Can you work these out from the drawing? Everything is in mm from the part's minimum corner. A direction names the side the tool comes from. Round coordinates to 2 decimals unless told otherwise and drop trailing zeros. Order: outer loops, then holes, each group sorted by start corner. A loop starts at its lowest first (then second) coordinate and runs counter-clockwise, first axis right, second up. Notation, with made-up numbers: (37.5, 69.5) - (56.5, 69.5) arc R29 ccw to (56.5, 104.5) - close; hole circle Ø10 at (-8, -18.5). An arc over 180 degrees is marked (long way). Write item = value, one per line.
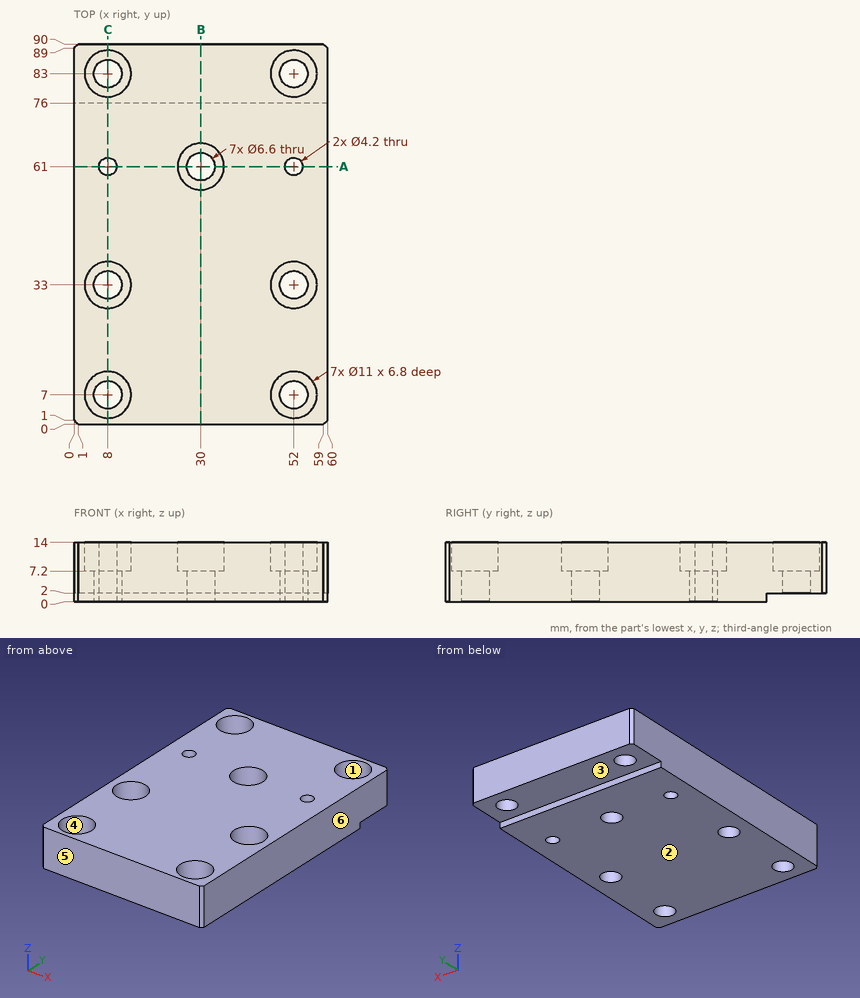
(1) If we section it at B-B (x = 30): Write out the boundary of the cut face in (y, z).
Computed:
outline = (0, 0) - (57.7, 0) - (57.7, 7.2) - (55.5, 7.2) - (55.5, 14) - (0, 14) - close; (64.3, 0) - (76, 0) - (76, 2) - (90, 2) - (90, 14) - (66.5, 14) - (66.5, 7.2) - (64.3, 7.2) - close
(2) Will these pins go through, and if not, where does the flat tip stop? P1, Ø12, axis at x = 32.5, y = 61.5, coming from the +Z side; P2, Ø7.5, axis at x = 52, y = 83, coming from the +Z side; P3, Ø0.6, axis at x = 32, z = 0.5, coming from the +Y side.
Computed:
P1 = 14
P2 = 7.2
P3 = 76
(3) On a 3-axis mill with a long thin cutter (end or side, diameter ignored), from which of +Z, -Z, +X, -X, +Y, -Y can I reach the whole of each face in a straight line? I mean the marked faces 1, 2 and 3. Say none if no direction works.
Computed:
face_1 = +Z
face_2 = -Z, +X, -X, +Y, -Y
face_3 = -Z, +X, -X, +Y
(4) Thinking about a two-plate mould opening in Y: for the marked faces 4, 5 and 6, which applies, +Y half, -Y half, draft (parallel to the pull), parting line (faces both ways), or undercut?
Computed:
face_4 = undercut
face_5 = -Y half
face_6 = draft
(5) If we section it at C-C (x = 8): State how many separate pieces and enclosed holes the cut face has, plus the area to 3 significant figures.
Computed:
separate_pieces = 5
enclosed_holes = 0
area = 819 mm^2
(6) If I drill on line 1 (Y direction, x = 8, z = 12.5); line 2 (Y direction, x = 8, z = 5.5); line 3 (X direction, y = 35.5, z = 11.25), over which ranges is the centre line in solid material (lowest first)? Write a range as from..to.
Computed:
line_1 = 0..1.5, 12.5..27.5, 38.5..58.9, 63.1..77.5, 88.5..90
line_2 = 0..3.7, 10.3..29.7, 36.3..58.9, 63.1..79.7, 86.3..90
line_3 = 0..3.1, 12.9..47.1, 56.9..60
(7) If we section it at A-A (y = 61): Write out the boundary of the cut face in (x, z).
Computed:
outline = (0, 0) - (5.9, 0) - (5.9, 14) - (0, 14) - close; (10.1, 0) - (26.7, 0) - (26.7, 7.2) - (24.5, 7.2) - (24.5, 14) - (10.1, 14) - close; (33.3, 0) - (49.9, 0) - (49.9, 14) - (35.5, 14) - (35.5, 7.2) - (33.3, 7.2) - close; (54.1, 0) - (60, 0) - (60, 14) - (54.1, 14) - close
